Drawing for the job (mm, zero at the part's lowest x, y, z). A direction names the side the tool comes from. Give positions to 0.01 mm unless a question says otherwise; leave off trailing zeros. Order: outer loops, then holes, each group sorted by start corner. A loop starts at its lowest first (then second) coordinate and runs counter-clockwise, first axis right, second up. Notation, with made-up numbers: (52, 51) - (93, 51) arc R29 cw to (93, 71) - close; hole circle Ø2 at (-37.5, 20). An arc over 180 degrees is marked (long way). Use a Markdown table: item, result. Add a question column.
(1) Slice it at B-B (z = 12.5). Write the cut outline in (x, y), then the cut area to 3 significant figures.
(2) Wall check: line 1 (Y direction, x = 9.5, z = 7.5); line 2 (X direction, y = 8.5, z = 7.5); line 3 (X direction, y = 71, z = 3.75). Give the ranges that are in metal, low to high.
(3) Which spindle directions (+Z, -Z, +X, -X, +Y, -Y) get a long thin tool onto all of the face, cutting with end or side? Do the marked faces 1 and 2. Say none if no direction does.
(4) Slice it at C-C (y = 109). Write the cut outline in (x, z), then the cut area to 3 significant figures.
(5) Slice it at A-A (y = 9). Write the cut outline in (x, z).
(6) Flat gauge pins, fed straight in: pin 1 (4 mm diameter, centred on x = 122.5, z = 7.5, fed in from +Y); pin 2 (8 mm diameter, centred on y = 75, z = 7.5, fed in from +X); pin 3 (4.5 mm diameter, centred on y = 30, z = 7.5, fed in from +X). Where does each tip first touch, or does it go through?
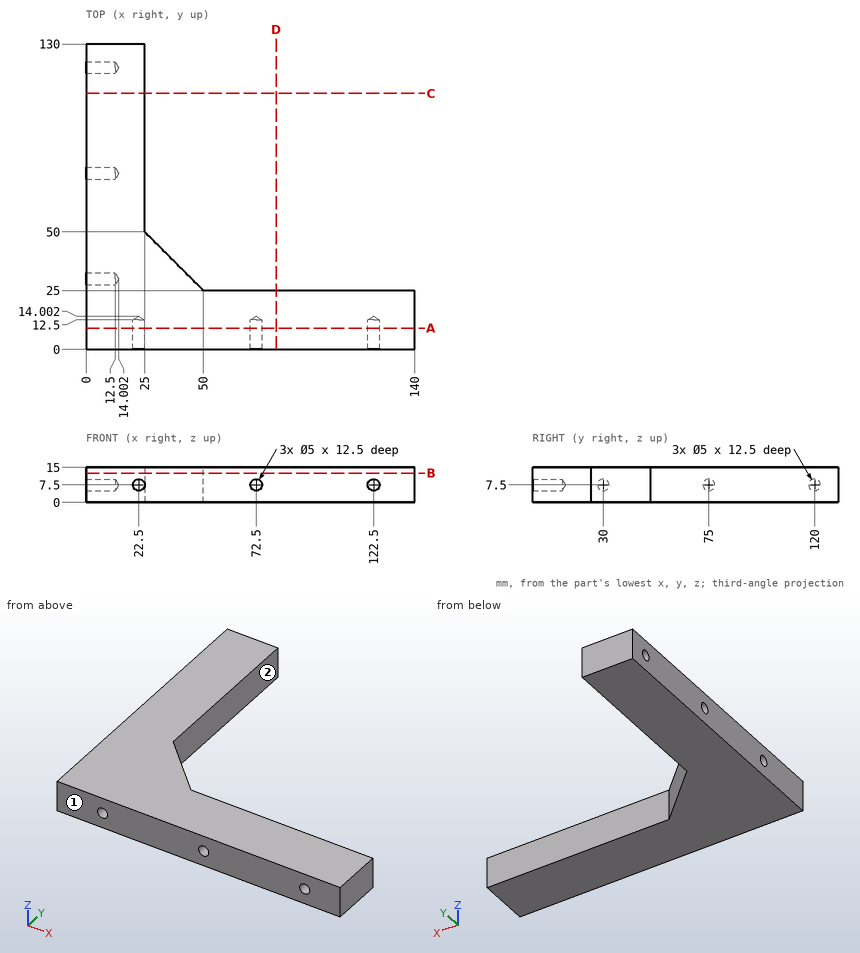
Solution:
| question | item | result |
|---|---|---|
| 1 | outline | (0, 0) - (140, 0) - (140, 25) - (50, 25) - (25, 50) - (25, 130) - (0, 130) - close |
| 1 | area | 6,440 mm2 |
| 2 | line 1 | 0 to 27.5, 32.5 to 72.5, 77.5 to 117.5, 122.5 to 130 |
| 2 | line 2 | 0 to 20, 25 to 70, 75 to 120, 125 to 140 |
| 2 | line 3 | 0 to 25 |
| 3 | face 1 | +Z, -Z, +X, -X, -Y |
| 3 | face 2 | +Z, -Z, +X, +Y |
| 4 | outline | (0, 0) - (25, 0) - (25, 15) - (0, 15) - close |
| 4 | area | 375 mm2 |
| 5 | outline | (0, 0) - (140, 0) - (140, 15) - (0, 15) - close; hole circle Ø5 at (22.5, 7.5); hole circle Ø5 at (72.5, 7.5); hole circle Ø5 at (122.5, 7.5) |
| 6 | pin 1 | y = 25 |
| 6 | pin 2 | x = 25 |
| 6 | pin 3 | x = 47.25 |
